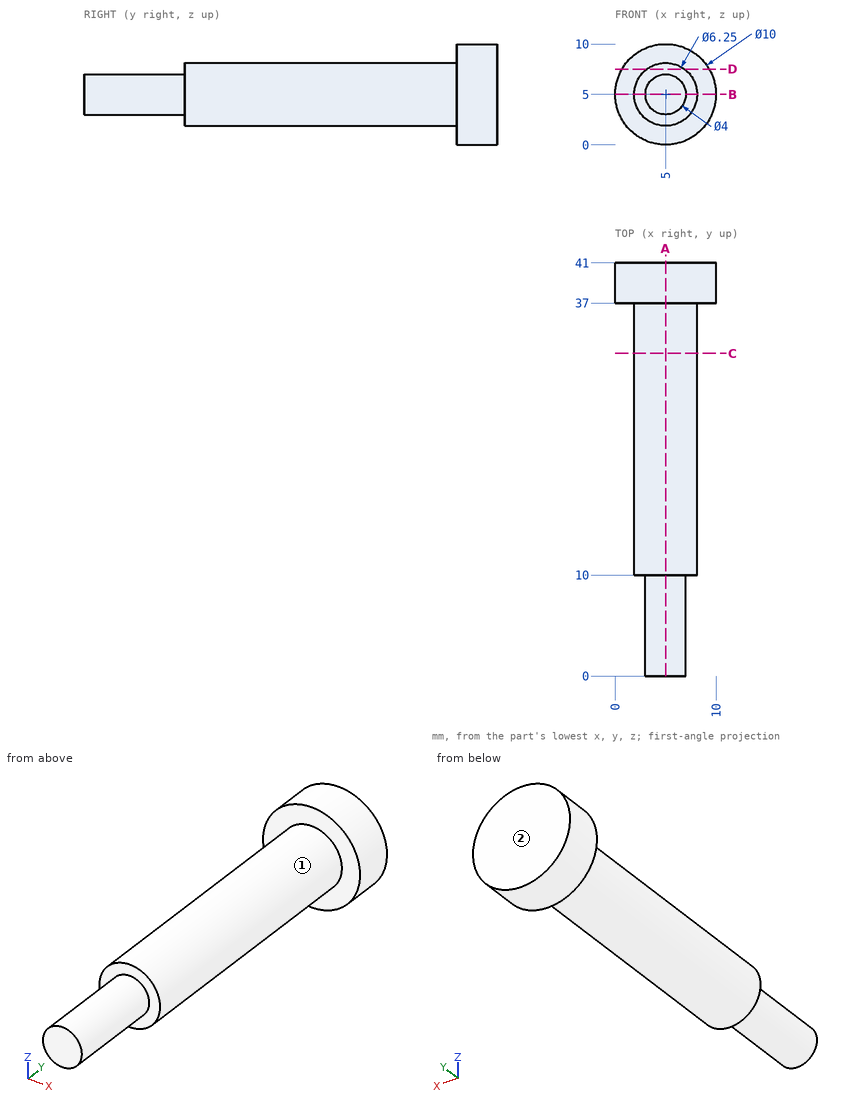
Geometry check sheet. Reference: drawing and pictorial views, mm from the part's lowest x, y, z. A direction names the side the tool comes from. Give positions to 0.01 mm unless a question says otherwise; leave off trailing zeros. Order: outer loops, then holes, each group sorted by start corner. A loop starts at its lowest first (then second) coordinate and runs counter-clockwise, first axis right, second up. Notation, with made-up numbers: (38.5, 68) - (97.5, 68) arc R11 cw to (97.5, 77) - close; hole circle Ø2 at (-4, -15.5). An arc over 180 degrees is marked (long way). Answer as CSV lines item,"result".
1. Section check D-D (z = 7.5). Record the boundary of the cut face in (x, y) (3 decimals), then the cut area to 3 significant figures.
Result sheet:
outline,"(0.67, 37) - (3.125, 37) - (3.125, 10) - (6.875, 10) - (6.875, 37) - (9.33, 37) - (9.33, 41) - (0.67, 41) - close"
area,"136 mm²"
2. Section check B-B (z = 5). Record the boundary of the cut face in (x, y) (3 decimals), then the cut area to 3 significant figures.
Result sheet:
outline,"(0, 37) - (1.875, 37) - (1.875, 10) - (3, 10) - (3, 0) - (7, 0) - (7, 10) - (8.125, 10) - (8.125, 37) - (10, 37) - (10, 41) - (0, 41) - close"
area,"249 mm²"
3. Section check C-C (y = 32). Record the boundary of the cut face in (x, z) (3 decimals), then the cut area to 3 significant figures.
Result sheet:
outline,"circle Ø6.25 at (5, 5)"
area,"30.7 mm²"
4. Tool access check on the marked faces 1 and 2. Record the directions out of +Z, -Z, +X, -X, +Y, -Y that give a thin tool (end or side, any length) a straight path to the whole face; none if there is none.
Result sheet:
face 1,"-Y"
face 2,"+Z, -Z, +X, -X, +Y"
5. Section check A-A (x = 5). Record the boundary of the cut face in (y, z) (3 decimals).
Result sheet:
outline,"(0, 3) - (10, 3) - (10, 1.875) - (37, 1.875) - (37, 0) - (41, 0) - (41, 10) - (37, 10) - (37, 8.125) - (10, 8.125) - (10, 7) - (0, 7) - close"
6. Scan lines: probe 1 along Y at (x, z) = (3, 6.5); probe 2 along Y at (x, z) = (1.5, 7.5); probe 3 along X at (y, z) = (34, 5.25). Record each from-to range of solid material in increasing order. Write a range as from..to.
Result sheet:
probe 1,"10..41"
probe 2,"37..41"
probe 3,"1.89..8.11"
7. Go/stop test with flat-tipped pins: P1, Ø5, axis at x = 1, z = 1, coming from the -Y side; P2, Ø2, axis at x = 6.5, y = 35.5, coming from the -Z side; P3, Ø6, axis at x = 4, y = 23, coming from the +Z side (3 decimals). Record where each tip stops, or that it passes through.
Result sheet:
P1,"y = 37"
P2,"z = 1.92"
P3,"z = 8.125"
